Here's how the part is built. I have some questions about the finished solid (model axes, mm). A direction names the side the tool comes from. Round coordinates to 2 decimals unless told otherwise and drop trailing zeros. Write each loop counter-clockwise with the first axis right and the second up, starting at its lowest first coordinate (ties: lowest second). Pieces come first, ordered by that corner, then holes. Notation, with made-up numbers: (-40, 89) -> (8, 89) arc R16 cw to (8, 117) -> close; hole circle Ø7 at (-12.5, -4). An arc over 180 degrees is marked (long way). Answer in a Markdown table with one row per item.
from build123d import *

# Parameters (mm, degrees)
CROSS_BLOCK_DEPTH      = 40
SIDE_LUG_DEPTH         = 20
BORE_26_SKETCH_R       = 13
BORE_26_DEPTH          = 20
CROSS_HOLE_20_SKETCH_R = 10
CROSS_HOLE_20_DEPTH    = 103.528044944


with BuildPart() as part:
    # Cross Profile Sketch → Cross Block (new body)
    with BuildSketch(Plane(origin=(0, 0, 0), x_dir=(1, 0, 0), z_dir=(0, 1, 0))):
        Polygon((0, 0), (20, 0), (20, 20), (56, 20), (56, 0), (76, 0), (76, -36), (56, -36), (56, -56), (20, -56), (20, -36), (0, -36), align=None)
    extrude(amount=CROSS_BLOCK_DEPTH)

    # Side Lug Sketch → Side Lug (add)
    with BuildSketch(Plane.XY.offset(56)):
        with BuildLine():
            Line((12.212406084, 28), (20, 28))
            Line((20, 28), (20, 40))
            ThreePointArc((20, 40), (14.32993543, 35.15273757), (12.212406084, 28))
        make_face()
        with BuildLine():
            Line((56, 40), (56, 28))
            Line((56, 28), (63.787593916, 28))
            ThreePointArc((63.787593916, 28), (61.67006457, 35.15273757), (56, 40))
        make_face()
        with BuildLine():
            Line((63.787593916, 12), (56, 12))
            Line((56, 12), (56, 0))
            ThreePointArc((56, 0), (63.15273757, 3.885057826), (63.787593916, 12))
        make_face()
        with BuildLine():
            Line((20, 0), (20, 12))
            Line((20, 12), (12.212406084, 12))
            ThreePointArc((12.212406084, 12), (12.84726243, 3.885057826), (20, 0))
        make_face()
    extrude(amount=-SIDE_LUG_DEPTH)

    # Bore Ø26 Sketch → Bore Ø26 (cut)
    with BuildSketch(Plane.XY.offset(56)):
        with Locations((38, 20)):
            Circle(BORE_26_SKETCH_R)
    extrude(amount=-BORE_26_DEPTH, mode=Mode.SUBTRACT)

    # Cross Hole Ø20 Sketch → Cross Hole Ø20 (cut, through all)
    with BuildSketch(Plane(origin=(76, 0, 0), x_dir=(0, 0, -1), z_dir=(1, 0, 0))):
        with Locations((-18, 20)):
            Circle(CROSS_HOLE_20_SKETCH_R)
    extrude(amount=-CROSS_HOLE_20_DEPTH, mode=Mode.SUBTRACT)


solid = part.part
1) We'd pull the mould along Y, two halves only. Please class faces 4 (the face through (61.73, 35.06, 46.14)), 5 (the face through (16, 28, 46)), 6 (the face through (63.09, 3.79, 46.14)): +Y half, -Y half, draft (parallel to the pull), parting line (faces both ways), or undercut.
Response:
| item | result |
|---|---|
| face 4 | +Y half |
| face 5 | undercut |
| face 6 | parting line |
2) I want a section at B-B, the plane x = 38. List the corners of the cut face in (y, z) for me.
Response:
| item | result |
|---|---|
| outline | (0, -20) -> (40, -20) -> (40, 56) -> (33, 56) -> (33, 36) -> (7, 36) -> (7, 56) -> (0, 56) -> close; hole circle Ø20 at (20, 18) |
3) For pin 1 (16 mm diameter, centred on y = 23, z = -11, fed in from -X); pin 2 (6 mm diameter, centred on x = 15.5, z = 41, fed in from -Y); pin 3 (10 mm diameter, centred on x = 10.5, y = 23.5, fed in from -Z); pin 4 (8.5 mm diameter, centred on x = 16, z = 43, fed in from +Y), each with a flat end and sliding along its axis, tell me the tip position at first contact or that it passes through.
Response:
| item | result |
|---|---|
| pin 1 | stops at x = 20 |
| pin 2 | stops at y = 0.13 |
| pin 3 | stops at z = 0 |
| pin 4 | stops at y = 40 |
4) I need wall thicknesses on line 1 (Y direction, x = 41, z = 18); line 2 (Y direction, x = 38, z = 51.25); line 3 (Z direction, x = 30, y = 29). Which ranges of each line are inside material? Lowest first, please. Write a range as [from, to].
Response:
| item | result |
|---|---|
| line 1 | y = [0, 10], [30, 40] |
| line 2 | y = [0, 7], [33, 40] |
| line 3 | z = [-20, 13.64], [22.36, 36] |
5) Which directions (+Z, -Z, +X, -X, +Y, -Y) give clear straight access to the entire face, cutting with the end or side of a thin tool? Please do faces 1 (the face through (56, 20, 46)), 2 (the face through (20, 20, -10)), 3 (the face through (14.388, 35.241, 46.14)).
Response:
| item | result |
|---|---|
| face 1 | +Z, +X |
| face 2 | -Z, -X, +Y, -Y |
| face 3 | +Z, -X, +Y |
6) I want a section at C-C, the plane y = 20. List the corners of the cut face in (x, z) for me, and give its area (3 significant figures).
Response:
| item | result |
|---|---|
| outline | (0, 0) -> (20, 0) -> (20, -20) -> (56, -20) -> (56, 0) -> (76, 0) -> (76, 8) -> (0, 8) -> close; (0, 28) -> (76, 28) -> (76, 36) -> (56, 36) -> (56, 56) -> (51, 56) -> (51, 36) -> (25, 36) -> (25, 56) -> (20, 56) -> (20, 36) -> (0, 36) -> close |
| area | 2,140 mm^2 |
7) I want a section at A-A, the plane z = 18. List the corners of the cut face in (x, y) for me.
Response:
| item | result |
|---|---|
| outline | (0, 0) -> (76, 0) -> (76, 10) -> (0, 10) -> close; (0, 30) -> (76, 30) -> (76, 40) -> (0, 40) -> close |
8) I want a section at D-D, the plane y = 3. List the corners of the cut face in (x, z) for me.
Response:
| item | result |
|---|---|
| outline | (0, 0) -> (20, 0) -> (20, -20) -> (56, -20) -> (56, 0) -> (76, 0) -> (76, 36) -> (62.49, 36) -> (62.49, 56) -> (13.51, 56) -> (13.51, 36) -> (0, 36) -> close |
